Can you work these out from the model? Positions are in its coordinate system, mm. A direction names the side the tool comes from. Give positions to 0.01 mm unless a question says otherwise; leave off trailing zeros. Loops run counter-clockwise (first coordinate to the right, second up) from the corner with the lowest first, then second, coordinate; pieces in that order, holes last. Notation, with made-up numbers: M 2.5,-22 L 44.5,-22 A22 cw 44.5,-11 Z; hole C 73.5,54 d3. An arc over 180 degrees is marked long. Use CSV: the item, a comma, the result in double quotes.
from build123d import *

# Parameters (mm, degrees)
SKETCH1_W                                    = 350
SKETCH1_H                                    = 110
BOSS_EXTRUDE1_DEPTH                          = 12
SKETCH2_W                                    = 350
SKETCH2_H                                    = 14
BOSS_EXTRUDE2_DEPTH                          = 120
CBORE_FOR_M8_HEXAGON_SOCKET_HEAD_CAP_2_COUNT = 2
CBORE_FOR_M8_HEXAGON_SOCKET_HEAD_CAP_2_PITCH = 65
CBORE_FOR_M8_HEXAGON_SOCKET_HEAD_CAP_3_COUNT = 2
CBORE_FOR_M8_HEXAGON_SOCKET_HEAD_CAP_3_PITCH = 300
CBORE_FOR_M8_HEXAGON_SOCKET_HEAD_CAP_4_COUNT = 2
CBORE_FOR_M8_HEXAGON_SOCKET_HEAD_CAP_4_PITCH = 306.960909563
CUT_EXTRUDE1_DEPTH                           = 230.804264538
CUT_EXTRUDE1_DEPTH_BACK                      = 230.804264538
SKETCH6_R                                    = 7
CUT_EXTRUDE2_DEPTH                           = 230.804264538
CUT_EXTRUDE2_DEPTH_BACK                      = 230.804264538
SKETCH7_R                                    = 12.5


with BuildPart() as part:
    # Sketch1 → Boss-Extrude1 (new body)
    with BuildSketch(Plane(origin=(0, 0, 0), x_dir=(1, 0, 0), z_dir=(0, 1, 0))):
        Rectangle(SKETCH1_W, SKETCH1_H)
    extrude(amount=BOSS_EXTRUDE1_DEPTH)

    # Sketch2 → Boss-Extrude2 (add)
    with BuildSketch(Plane(origin=(0, 12, 0), x_dir=(1, 0, 0), z_dir=(0, 1, 0))):
        with Locations((0, 7)):
            Rectangle(SKETCH2_W, SKETCH2_H)
    extrude(amount=BOSS_EXTRUDE2_DEPTH)

    # Sketch4 → CBORE for M8 Hexagon socket head cap screws1 (revolve, cut)
    with BuildSketch(Plane(origin=(-150, 12, -32.5), x_dir=(0, 0, 1), z_dir=(1, 0, 0))):
        Polygon((0, 0), (0, 15.103872786), (4.5, 12.4), (4.5, 9), (7.5, 9), (7.5, 0.025), (7.525, 0), align=None)
    cbore_for_m8_hexagon_socket_head_cap_scr = revolve(axis=Axis((-150, 18.35, -32.5), (0, -1, 0)), mode=Mode.SUBTRACT)

    # CBORE for M8 Hexagon socket head cap 2: CBORE for M8 Hexagon socket head cap screws1 ×2
    with Locations(*[(0, 0, i * CBORE_FOR_M8_HEXAGON_SOCKET_HEAD_CAP_2_PITCH) for i in range(1, CBORE_FOR_M8_HEXAGON_SOCKET_HEAD_CAP_2_COUNT)]):
        add(cbore_for_m8_hexagon_socket_head_cap_scr, mode=Mode.SUBTRACT)

    # CBORE for M8 Hexagon socket head cap 3: CBORE for M8 Hexagon socket head cap screws1 ×2
    with Locations(*[(i * CBORE_FOR_M8_HEXAGON_SOCKET_HEAD_CAP_3_PITCH, 0, 0) for i in range(1, CBORE_FOR_M8_HEXAGON_SOCKET_HEAD_CAP_3_COUNT)]):
        add(cbore_for_m8_hexagon_socket_head_cap_scr, mode=Mode.SUBTRACT)

    # CBORE for M8 Hexagon socket head cap 4: CBORE for M8 Hexagon socket head cap screws1 ×2
    with Locations(*[Vector(0.9773231400267972, 0, 0.21175334700580606) * (i * CBORE_FOR_M8_HEXAGON_SOCKET_HEAD_CAP_4_PITCH) for i in range(1, CBORE_FOR_M8_HEXAGON_SOCKET_HEAD_CAP_4_COUNT)]):
        add(cbore_for_m8_hexagon_socket_head_cap_scr, mode=Mode.SUBTRACT)

    # Sketch6 → Cut-Extrude1 (cut, two sides: drawn at the far end of the back side and taken through both)
    with BuildSketch(Plane(origin=(0, 0, -14), x_dir=(-1, 0, 0), z_dir=(0, 0, -1)).offset(-CUT_EXTRUDE1_DEPTH_BACK)):
        with Locations((95, 82)):
            Circle(SKETCH6_R)
    extrude(amount=CUT_EXTRUDE1_DEPTH + CUT_EXTRUDE1_DEPTH_BACK, mode=Mode.SUBTRACT)

    # Sketch7 → Cut-Extrude2 (cut, two sides: drawn at the far end of the back side and taken through both)
    with BuildSketch(Plane(origin=(0, 0, -14), x_dir=(-1, 0, 0), z_dir=(0, 0, -1)).offset(-CUT_EXTRUDE2_DEPTH_BACK)):
        with Locations((-65, 82)):
            Circle(SKETCH7_R)
    extrude(amount=CUT_EXTRUDE2_DEPTH + CUT_EXTRUDE2_DEPTH_BACK, mode=Mode.SUBTRACT)


solid = part.part
Q1. I want a section at D-D, the plane x = -150. Please give me the cut outline in (y, z) (3 decimals), then the cut area to 3 significant figures.
Model answer:
outline,"M 0,-55 L 12,-55 L 12,-40.025 L 11.975,-40 L 3,-40 L 3,-37 L 0,-37 Z; M 0,-28 L 3,-28 L 3,-25 L 11.975,-25 L 12,-24.975 L 12,-14 L 132,-14 L 132,0 L 12,0 L 12,24.975 L 11.975,25 L 3,25 L 3,28 L 0,28 Z; M 0,37 L 3,37 L 3,40 L 11.975,40 L 12,40.025 L 12,55 L 0,55 Z"
area,"2,680 mm2"
Q2. I want a section at C-C, the plane x = 65. Please give me the cut outline in (y, z), then the cut area to 3 significant figures.
Model answer:
outline,"M 0,-55 L 12,-55 L 12,-14 L 69.5,-14 L 69.5,0 L 12,0 L 12,55 L 0,55 Z; M 94.5,-14 L 132,-14 L 132,0 L 94.5,0 Z"
area,"2,650 mm2"
Q3. For faces 4 (the cylindrical face through (154.39, 1.52, -33.48)), 5 (the flat face through (-2, 71, -14)), 6 (the cylindrical face through (150, 8, 25)), which set-ups out of +Z, -Z, +X, -X, +Y, -Y let a thin tool reach every point of the face, with its end or its side?
Model answer:
face 4,"+Y, -Y"
face 5,"-Z, +X, -X, +Y"
face 6,"+Y"
Q4. I want a section at B-B, the plane y = 82. Please give me the cut outline in (x, z), then the cut area to 3 significant figures.
Model answer:
outline,"M -175,-14 L -102,-14 L -102,0 L -175,0 Z; M -88,-14 L 52.5,-14 L 52.5,0 L -88,0 Z; M 77.5,-14 L 175,-14 L 175,0 L 77.5,0 Z"
area,"4,350 mm2"
Q5. I want a section at A-A, the plane z = -32.5. Please give me the cut outline in (x, y) (3 decimals).
Model answer:
outline,"M -175,0 L -154.5,0 L -154.5,3 L -157.5,3 L -157.5,11.975 L -157.525,12 L -175,12 Z; M -145.5,0 L 145.5,0 L 145.5,3 L 142.5,3 L 142.5,11.975 L 142.475,12 L -142.475,12 L -142.5,11.975 L -142.5,3 L -145.5,3 Z; M 154.5,0 L 175,0 L 175,12 L 157.525,12 L 157.5,11.975 L 157.5,3 L 154.5,3 Z"
Q6. If we mould it in two halves opening along X, with no side actions, what happens to faces 1 (the cylindrical face through (66.627, 94.394, -6.902)), 2 (the flat face through (175, 36, -4)), 3 (the flat face through (-2, 12, 27))? For each: released by +X, released by -X, zero draft, split by the parting line, or undercut.
Model answer:
face 1,"undercut"
face 2,"released by +X"
face 3,"zero draft"
Q7. Please list where these lines run through material, in increasing order: L1, parallel to X at y = 0.75, z = 32.5; L2, parallel to X at y = 6.75, z = -32.5; L3, parallel to Z at x = -150, y = 8. Write a range as from..to.
Model answer:
L1,"-175..-154.5, -145.5..145.5, 154.5..175"
L2,"-175..-157.5, -142.5..142.5, 157.5..175"
L3,"-55..-40, -25..25, 40..55"
Q8. I'm going to push flat-ended pins straight in: P1, Ø8, axis at x = 21.5, y = 107, coming from the +Z side; P2, Ø17, axis at x = 150, z = -32.5, coming from the -Y side; P3, Ø12, axis at x = 153.5, z = 29, coming from the +Y side; P4, Ø4.5, axis at x = -151, z = 29.5, coming from the +Y side. Where does each tip first touch, or does it pass through?
Model answer:
P1,"z = 0"
P2,"y = 0"
P3,"y = 12"
P4,"y = 3"
